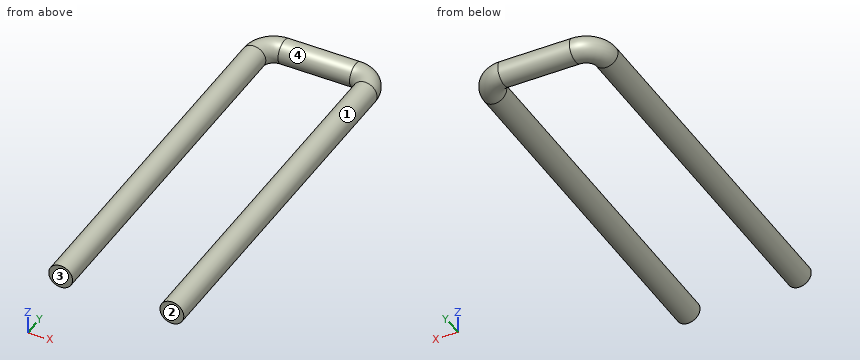
```python
from build123d import *

# Parameters (mm, degrees)
SKETCH_2_R = 3


with BuildPart() as part:
    # 扫描1: sweep along a path in 草图1
    with BuildLine(Plane.XY) as sweep_1_path:
        Line((-14, 0), (-14, 91))
        ThreePointArc((-14, 91), (-12.535533906, 94.535533906), (-9, 96))
        Line((-9, 96), (9, 96))
        ThreePointArc((9, 96), (12.535533906, 94.535533906), (14, 91))
        Line((14, 91), (14, 0))
    # 草图2 → 扫描1 (sweep)
    with BuildSketch(Plane(origin=(0, 0, 0), x_dir=(1, 0, 0), z_dir=(0, 1, 0))):
        with Locations((-14, 0)):
            Circle(SKETCH_2_R)
    sweep(path=sweep_1_path.line)


solid = part.part
```
Could you check a few things on this model? Use its own coordinates, in mm. Face numbers are marked on the shaded views. A direction names the side the tool comes from. Round coordinates to 2 decimals unless told otherwise and drop trailing zeros. Loops run counter-clockwise (first coordinate to the right, second up) from the corner with the lowest first, then second, coordinate; pieces in that order, holes last. Notation, with made-up numbers: (27, 49.25) - (69, 49.25) arc R25 cw to (69, 71.25) - close; hole circle Ø5 at (-10, 66). An arc over 180 degrees is marked (long way). Use CSV: the item, a comma, the result in double quotes.
Item 1: If we section it at B-B on y = 38: List the corners of the cut face in (x, z) for me.
Here are the results:
outline,"circle Ø6 at (-14, 0); circle Ø6 at (14, 0)"
Item 2: I need wall thicknesses on L1, parallel to X at y = 85, z = 0.5; L2, parallel to X at y = 54.5, z = 1.5; L3, parallel to Y at x = -11.5, z = -1.5 (3 decimals). Which ranges of each line are inside material? Lowest first, please. Write a range as [from, to].
Here are the results:
L1,"x = [-16.96, -11.04], [11.04, 16.96]"
L2,"x = [-16.6, -11.4], [11.4, 16.6]"
L3,"y = [0, 98.175]"
Item 3: Will these pins go through, and if not, where does the flat tip stop? pin 1 (1.5 mm diameter, centred on x = -6.5, z = -2, fed in from -Y); pin 2 (1.5 mm diameter, centred on y = 63.5, z = -2, fed in from -X).
Here are the results:
pin 1,"stops at y = 93.27"
pin 2,"stops at x = -16.73"
Item 4: If we section it at A-A on z = 0: List the corners of the cut face in (x, y) for me, then the cut area to 3 significant figures.
Here are the results:
outline,"(-17, 0) - (-11, 0) - (-11, 91) arc R2 cw to (-9, 93) - (9, 93) arc R2 cw to (11, 91) - (11, 0) - (17, 0) - (17, 91) arc R8 ccw to (9, 99) - (-9, 99) arc R8 ccw to (-17, 91) - close"
area,"1,290 mm²"
Item 5: For the marked faces 1 and 2, which set-ups out of +Z, -Z, +X, -X, +Y, -Y let a thin tool reach every point of the face, with its end or its side?
Here are the results:
face 1,"-Y"
face 2,"+Z, -Z, +X, -X, -Y"
Item 6: If we section it at C-C on x = 2: List the corners of the cut face in (y, z) for me, then the cut area to 3 significant figures.
Here are the results:
outline,"circle Ø6 at (96, 0)"
area,"28.3 mm²"
Item 7: If we mould it in two halves opening along X, with no side actions, what happens to the marked faces 3 and 4? For each: pulls with the +X half, pulls with the -X half, needs draft (parallel to the pull), parting line crosses it, or undercut.
Here are the results:
face 3,"needs draft"
face 4,"undercut"
